Work out the finished part from the listing and answer in its coordinate system (mm). A direction names the side the tool comes from. Give positions to 0.01 mm unless a question says otherwise; leave off trailing zeros. Write each loop counter-clockwise with the first axis right and the second up, starting at its lowest first coordinate (ties: lowest second). Pieces come first, ordered by that corner, then holes.
1) A tool of negligible diameter and unlimited length cuts with its end or side. For faces 1 (the face through (-5.58, 19.93, 9.48)), 2 (the face through (3.2, 7.9, -10)), from which of +Z, -Z, +X, -X, +Y, -Y can it reach the whole face along a straight path? Write none if from no direction.
2) Find section A-A (z = 0). Determine the outline of the cut face in (x, y), plus the area to 4 significant figures.
3) Straight lines are drawn through the part: probe 1 along X at (y, z) = (18.5, 0); probe 2 along X at (y, z) = (9.75, 0); probe 3 along Z at (x, y) = (0.75, 8). For each, find the intervals that lie inside material, in ascending order.
4) Find section B-B (y = 10). Determine the outline of the cut face in (x, z), plus the area to 3 significant figures.
5) Determine the mould class of faces 3 (the face through (-6.6, 15, -8.4)), 4 (the face through (-5.423, 19.93, -9.571)), 5 (the face through (3.584, 12.325, -2.285)) for opening direction Z: pulls with the +Z half, pulls with the -Z half, needs draft (parallel to the pull), parting line crosses it, or undercut.
6) Given pin 1 Ø2 at (y, z) = (20, 7.5) entering from +X; pin 2 Ø2 at (y, z) = (12.5, -8.5) entering from -X; pin 3 Ø10 at (y, z) = (8, -1) entering from +X, each flat-ended and moving along its own axis, determine where each tip first touches the part or whether it passes through.
```python
from build123d import *

# Parameters (mm, degrees)
BOSS_EXTRUDE1_DEPTH = 25
SKETCH3_OUTSIDE_W   = 32.376
SKETCH3_OUTSIDE_H   = 35.78
SKETCH3_OUTSIDE_R   = 10.5
CUT_EXTRUDE1_DEPTH  = 15
CHAMFER1_SIZE       = 1
M10_TAPPED_HOLE1_D  = 8.5


with BuildPart() as part:
    # Sketch1 → Boss-Extrude1 (new body)
    with BuildSketch(Plane(origin=(0, 0, 0), x_dir=(1, 0, 0), z_dir=(0, 1, 0))):
        Polygon((11, -6.350852961), (11, 6.350852961), (0, 12.701705922), (-11, 6.350852961), (-11, -6.350852961), (0, -12.701705922), align=None)
    extrude(amount=BOSS_EXTRUDE1_DEPTH)

    # Sketch3 outside → Cut-Extrude1 (cut)
    with BuildSketch(Plane.XZ):
        Rectangle(SKETCH3_OUTSIDE_W, SKETCH3_OUTSIDE_H)
        with Locations(Location((0, 0, 0), (0, 0, 270))):
            Circle(SKETCH3_OUTSIDE_R, mode=Mode.SUBTRACT)
    extrude(amount=-CUT_EXTRUDE1_DEPTH, mode=Mode.SUBTRACT)

    # Chamfer1
    chamfer1_edges = [part.edges().sort_by_distance(p)[0] for p in [
        (0, 0, 10.5),
    ]]
    chamfer(chamfer1_edges, length=CHAMFER1_SIZE)

    # M10 Tapped Hole1 (through all)
    with Locations(Plane.ZX.offset(25)):
        with Locations((0, 0)):
            Hole(M10_TAPPED_HOLE1_D / 2)


solid = part.part
```
Results:
1. face 1: +Z, -X, +Y, -Y
1. face 2: -Y
2. outline: (-11, 15) - (-10.5, 15) - (-10.5, 1) - (-9.5, 0) - (-4.25, 0) - (-4.25, 25) - (-11, 25) - close; (4.25, 0) - (9.5, 0) - (10.5, 1) - (10.5, 15) - (11, 15) - (11, 25) - (4.25, 25) - close
2. area: 321.5 mm2
3. probe 1: x = -11 to -4.25, 4.25 to 11
3. probe 2: x = -10.5 to -4.25, 4.25 to 10.5
3. probe 3: z = -10.47 to -4.18, 4.18 to 10.47
4. outline: circle Ø21 at (0, 0); hole circle Ø8.5 at (0, 0)
4. area: 290 mm2
5. face 3: needs draft
5. face 4: pulls with the -Z half
5. face 5: undercut
6. pin 1: stops at x = 10.74
6. pin 2: stops at x = -7.35
6. pin 3: stops at x = 10.5
